Here's how the part is built. I have some questions about the finished solid (model axes, mm). Coordinates: 2 decimals unless noted, no trailing zeros. Loops run counter-clockwise (first coordinate to the right, second up) from the corner with the lowest first, then second, coordinate; pieces in that order, holes last. Notation, with made-up numbers: M 71.5,13 L 130.5,13 A23 ccw 130.5,39 Z; hole C 81.5,13 d7. An arc over 180 degrees is marked long. Use one line per item in the form item = value. Start each with the question number.
(1) Imagine slicing it at B-B, the plane y = 0. Please give me the cut outline in (x, z), and give its area (3 significant figures).
(2) Please list where these lines run through material, in increasing order: L1, parallel to Y at x = 14, z = -250; L2, parallel to Z at x = 19, y = -4.
(3) Thinking about a two-plate mould opening in Z: for faces 1 (the cylindrical face through (9.86, -3.83, 240.763)), 2 (the flat face through (10, 65, 5)), 3 (the flat face through (10, -1, -350)), which applies, +Z half, -Z half, draft (parallel to the pull), parting line (faces both ways), or undercut?
(4) Imagine slicing it at A-A, the plane z = -250. Please give me the cut outline in (x, y).
```python
from build123d import *

# Parameters (mm, degrees)
SKETCH1_W           = 700
SKETCH1_H           = 130
SKETCH1_R           = 10
BOSS_EXTRUDE1_DEPTH = 20


with BuildPart() as part:
    # Sketch1 → Boss-Extrude1 (new body)
    with BuildSketch(Plane(origin=(0, 0, 0), x_dir=(0, 0, -1), z_dir=(1, 0, 0))):
        Rectangle(SKETCH1_W, SKETCH1_H)
        with Locations((-250, 0)):
            Circle(SKETCH1_R, mode=Mode.SUBTRACT)
        with Locations((250, 0)):
            Circle(SKETCH1_R, mode=Mode.SUBTRACT)
    extrude(amount=BOSS_EXTRUDE1_DEPTH)


solid = part.part
```
Answer:
q1.outline = M 0,-350 L 20,-350 L 20,-260 L 0,-260 Z; M 0,-240 L 20,-240 L 20,240 L 0,240 Z; M 0,260 L 20,260 L 20,350 L 0,350 Z
q1.area = 13,200 mm²
q2.L1 = -65 to -10, 10 to 65
q2.L2 = -350 to -259.17, -240.83 to 240.83, 259.17 to 350
q3.face_1 = undercut
q3.face_2 = draft
q3.face_3 = -Z half
q4.outline = M 0,-65 L 20,-65 L 20,-10 L 0,-10 Z; M 0,10 L 20,10 L 20,65 L 0,65 Z
